Verification items for the finished model (mm, model axes). A direction names the side the tool comes from. Give positions to 0.01 mm unless a question says otherwise; leave off trailing zeros. Loops run counter-clockwise (first coordinate to the right, second up) from the corner with the lowest first, then second, coordinate; pieces in that order, holes last. Notation, with made-up numbers: (-13, 65.5) - (21, 65.5) arc R18 cw to (21, 84.5) - close; hole circle Ø4 at (-21, 35.25). An arc over 180 degrees is marked (long way). One line per question, with ' | ' between items. Start each with the question number.
1. Section check D-D, the plane x = 273. Enter the section's corners in (y, z).
2. Section check C-C, the plane x = 74. Enter the section's corners in (y, z).
3. Section check A-A, the plane z = -28.5. Enter the section's corners in (x, y).
4. Mould release check, pull along Z, two halves, no side actions. Record for faces 1 (the face through (200, -21, -1)), 2 (the face through (10, 2, -53)), 3 (the face through (3.01, 1.48, -57.15)): +Z half, -Z half, draft (parallel to the pull), parting line (faces both ways), or undercut.
5. Section check B-B, the plane y = -25.5. Enter the section's corners in (x, z), then the cut area to 3 significant figures.
6. Thickness scan on line 1 along Z through (x, y) = (299.2, -15); line 2 along Y through (x, z) = (51, 25); line 3 along X through (y, z) = (-33, 10.5). Record the ranges inside material, lowest first. Write a range as from..to.
7. Tool access check on faces 4 (the face through (110, 2, -53)), 5 (the face through (297, -23, -1)), 6 (the face through (65, 0, -1)). Record the directions out of +Z, -Z, +X, -X, +Y, -Y that give a thin tool (end or side, any length) a straight path to the whole face; none if there is none.
8. Depth check by flat-ended pin: pin 1 Ø5.5 at (y, z) = (-15, 35) entering from -X; pin 2 Ø7 at (x, z) = (110, -50) entering from -Y; pin 3 Ø5.5 at (y, z) = (-31, 35) entering from -X; pin 4 Ø10 at (x, y) = (173.5, -9.5) entering from +Z. Enter the tip coordinate at first touch or a pass-through.
from build123d import *

# Parameters (mm, degrees)
EXTRUDE_1_DEPTH      = 60
EXTRUDE_1_DEPTH_BACK = 60
CUT_EXTRUDE_1_DEPTH  = 310.232921921
FILLET_1_R           = 10
CUT_EXTRUDE_2_REACH  = 311.233
SKETCH_3_R           = 3
CUT_EXTRUDE_3_REACH  = 310.811
SKETCH_4_R           = 2.1


with BuildPart() as part:
    # 草图1 → 拉伸-薄壁1 (new, two sides: drawn at the far end of the back side and taken through both)
    with BuildSketch(Plane.XY.offset(-EXTRUDE_1_DEPTH_BACK)):
        Polygon((0, 0), (170, 0), (230, -42), (300, -42), (300, -7), (297, -7), (297, -39), (230.945666692, -39), (170.945666692, 3), (0, 3), align=None)
    extrude(amount=EXTRUDE_1_DEPTH + EXTRUDE_1_DEPTH_BACK)

    # 草图2 → 切除-拉伸1 (cut, through all)
    with BuildSketch(Plane(origin=(0, 3, 0), x_dir=(1, 0, 0), z_dir=(0, 1, 0))):
        Polygon((120, 60), (120, 35), (170.945666692, 35), (297, 60), align=None)
        Polygon((297, -60), (120, -60), (120, -35), (170.945666692, -35), align=None)
    extrude(amount=-CUT_EXTRUDE_1_DEPTH, mode=Mode.SUBTRACT)

    # 圆角1
    fillet_1_edges = [part.edges().sort_by_distance(p)[0] for p in [
        (0, 1.5, -60),
        (0, 1.5, 60),
        (120, 1.5, -60),
        (120, 1.5, 60),
    ]]
    fillet(fillet_1_edges, radius=FILLET_1_R)

    # 草图3 → 切除-拉伸2 (cut, up to next)
    with BuildSketch(Plane(origin=(0, 3, 0), x_dir=(1, 0, 0), z_dir=(0, 1, 0)), mode=Mode.PRIVATE) as cut_extrude_2_sk1:
        with Locations(Location((10, 50, 0), (0, 0, 270))):
            Circle(SKETCH_3_R)
    cut_extrude_2_tool1 = extrude(cut_extrude_2_sk1.sketch, amount=-CUT_EXTRUDE_2_REACH, mode=Mode.PRIVATE) & part.part
    # 草图3 → 切除-拉伸2 (cut, up to next)
    with BuildSketch(Plane(origin=(0, 3, 0), x_dir=(1, 0, 0), z_dir=(0, 1, 0)), mode=Mode.PRIVATE) as cut_extrude_2_sk2:
        with Locations(Location((110, 50, 0), (0, 0, 270))):
            Circle(SKETCH_3_R)
    cut_extrude_2_tool2 = extrude(cut_extrude_2_sk2.sketch, amount=-CUT_EXTRUDE_2_REACH, mode=Mode.PRIVATE) & part.part
    # 草图3 → 切除-拉伸2 (cut, up to next)
    with BuildSketch(Plane(origin=(0, 3, 0), x_dir=(1, 0, 0), z_dir=(0, 1, 0)), mode=Mode.PRIVATE) as cut_extrude_2_sk3:
        with Locations(Location((110, -50, 0), (0, 0, 270))):
            Circle(SKETCH_3_R)
    cut_extrude_2_tool3 = extrude(cut_extrude_2_sk3.sketch, amount=-CUT_EXTRUDE_2_REACH, mode=Mode.PRIVATE) & part.part
    # 草图3 → 切除-拉伸2 (cut, up to next)
    with BuildSketch(Plane(origin=(0, 3, 0), x_dir=(1, 0, 0), z_dir=(0, 1, 0)), mode=Mode.PRIVATE) as cut_extrude_2_sk4:
        with Locations(Location((10, -50, 0), (0, 0, 270))):
            Circle(SKETCH_3_R)
    cut_extrude_2_tool4 = extrude(cut_extrude_2_sk4.sketch, amount=-CUT_EXTRUDE_2_REACH, mode=Mode.PRIVATE) & part.part
    add(cut_extrude_2_tool1.solids().sort_by_distance((10, 3, -50))[0], mode=Mode.SUBTRACT)
    add(cut_extrude_2_tool2.solids().sort_by_distance((110, 3, -50))[0], mode=Mode.SUBTRACT)
    add(cut_extrude_2_tool3.solids().sort_by_distance((110, 3, 50))[0], mode=Mode.SUBTRACT)
    add(cut_extrude_2_tool4.solids().sort_by_distance((10, 3, 50))[0], mode=Mode.SUBTRACT)

    # 草图4 → 切除-拉伸3 (cut, up to next)
    with BuildSketch(Plane(origin=(300, 0, 0), x_dir=(0, 0, -1), z_dir=(1, 0, 0)), mode=Mode.PRIVATE) as cut_extrude_3_sk1:
        with Locations(Location((-35, -15, 0), (0, 0, 90))):
            Circle(SKETCH_4_R)
    cut_extrude_3_tool1 = extrude(cut_extrude_3_sk1.sketch, amount=-CUT_EXTRUDE_3_REACH, mode=Mode.PRIVATE) & part.part
    # 草图4 → 切除-拉伸3 (cut, up to next)
    with BuildSketch(Plane(origin=(300, 0, 0), x_dir=(0, 0, -1), z_dir=(1, 0, 0)), mode=Mode.PRIVATE) as cut_extrude_3_sk2:
        with Locations(Location((-35, -31, 0), (0, 0, 90))):
            Circle(SKETCH_4_R)
    cut_extrude_3_tool2 = extrude(cut_extrude_3_sk2.sketch, amount=-CUT_EXTRUDE_3_REACH, mode=Mode.PRIVATE) & part.part
    # 草图4 → 切除-拉伸3 (cut, up to next)
    with BuildSketch(Plane(origin=(300, 0, 0), x_dir=(0, 0, -1), z_dir=(1, 0, 0)), mode=Mode.PRIVATE) as cut_extrude_3_sk3:
        with Locations(Location((35, -31, 0), (0, 0, 90))):
            Circle(SKETCH_4_R)
    cut_extrude_3_tool3 = extrude(cut_extrude_3_sk3.sketch, amount=-CUT_EXTRUDE_3_REACH, mode=Mode.PRIVATE) & part.part
    # 草图4 → 切除-拉伸3 (cut, up to next)
    with BuildSketch(Plane(origin=(300, 0, 0), x_dir=(0, 0, -1), z_dir=(1, 0, 0)), mode=Mode.PRIVATE) as cut_extrude_3_sk4:
        with Locations(Location((35, -15, 0), (0, 0, 90))):
            Circle(SKETCH_4_R)
    cut_extrude_3_tool4 = extrude(cut_extrude_3_sk4.sketch, amount=-CUT_EXTRUDE_3_REACH, mode=Mode.PRIVATE) & part.part
    add(cut_extrude_3_tool1.solids().sort_by_distance((300, -15, 35))[0], mode=Mode.SUBTRACT)
    add(cut_extrude_3_tool2.solids().sort_by_distance((300, -31, 35))[0], mode=Mode.SUBTRACT)
    add(cut_extrude_3_tool3.solids().sort_by_distance((300, -31, -35))[0], mode=Mode.SUBTRACT)
    add(cut_extrude_3_tool4.solids().sort_by_distance((300, -15, -35))[0], mode=Mode.SUBTRACT)


solid = part.part
Results list:
1) outline: (-42, -55.24) - (-39, -55.24) - (-39, 55.24) - (-42, 55.24) - close
2) outline: (0, -60) - (3, -60) - (3, 60) - (0, 60) - close
3) outline: (0, 0) - (170, 0) - (230, -42) - (300, -42) - (300, -7) - (297, -7) - (297, -39) - (230.95, -39) - (170.95, 3) - (0, 3) - close
4) face 1: draft | face 2: undercut | face 3: -Z half
5) outline: (206.43, -42.04) - (211.66, -43.07) - (211.66, 43.07) - (206.43, 42.04) - close; (297, -60) - (300, -60) - (300, 60) - (297, 60) - close | area: 805 mm²
6) line 1: -60..-37.1, -32.9..32.9, 37.1..60 | line 2: 0..3 | line 3: 217.14..222.37, 297..300
7) face 4: +Y, -Y | face 5: +Z, -Z, +Y | face 6: +Z, -Z, -X, -Y
8) pin 1: x = 187.5 | pin 2: y = 0 | pin 3: x = 210.36 | pin 4: through
